Job drawing, mm, ordinate dimensions from the low corner. One solid piece. Round coordinates to 2 decimals unless told otherwise and drop trailing zeros. Order: outer loops, then holes, each group sorted by start corner. A loop starts at its lowest first (then second) coordinate and runs counter-clockwise, first axis right, second up. Notation, with made-up numbers: M 41,70.5 L 86,70.5 A13 ccw 86,84.5 Z; hole C 39.5,59 d1. An arc over 180 degrees is marked long. Answer as a JSON object with one key per item and string values. Group by question number.
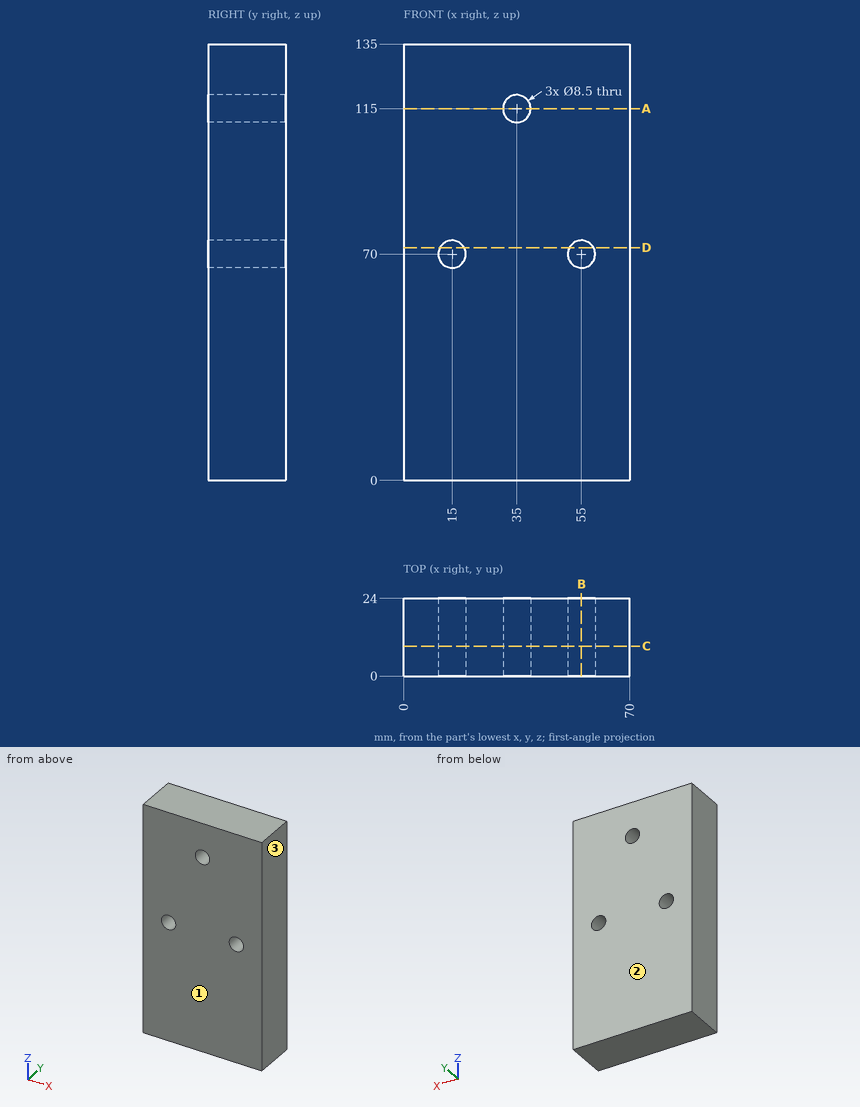
Item 1: Flat gauge pin, fed straight in: pin 1 Ø10 at (x, z) = (55, 70) entering from +Y. Where does the tip first touch, or does it go through?
Item 2: Two-plate mould, pull along Y, no slides. Class the marked faces 1, 2 and 3: +Y half, -Y half, draft (parallel to the pull), parting line (faces both ways), or undercut.
Item 3: Cut at D-D, the plane z = 72. Give the cut face in (x, y), and give its area (3 significant figures).
Item 4: Drill centre lines: line 1 (X direction, y = 11.5, z = 70); line 2 (Z direction, x = 55, y = 16); line 3 (Z direction, x = 34.5, y = 20.25). Where is each one in solid material? Low to high. Write a range as [from, to].
Item 5: Cut at A-A, the plane z = 115. Give the cut face in (x, y).
Item 6: Cut at C-C, the plane y = 9.25. Give the cut face in (x, z).
Item 7: Cut at B-B, the plane x = 55. Give the cut face in (y, z), and give its area (3 significant figures).
Response values:
{
 "1": {"pin 1": "y = 24"},
 "2": {"face 1": "-Y half", "face 2": "+Y half", "face 3": "draft"},
 "3": {"outline": "M 0,0 L 11.25,0 L 11.25,24 L 0,24 Z; M 18.75,0 L 51.25,0 L 51.25,24 L 18.75,24 Z; M 58.75,0 L 70,0 L 70,24 L 58.75,24 Z", "area": "1,320 mm^2"},
 "4": {"line 1": "[0, 10.75], [19.25, 50.75], [59.25, 70]", "line 2": "[0, 65.75], [74.25, 135]", "line 3": "[0, 110.78], [119.22, 135]"},
 "5": {"outline": "M 0,0 L 30.75,0 L 30.75,24 L 0,24 Z; M 39.25,0 L 70,0 L 70,24 L 39.25,24 Z"},
 "6": {"outline": "M 0,0 L 70,0 L 70,135 L 0,135 Z; hole C 15,70 d8.5; hole C 35,115 d8.5; hole C 55,70 d8.5"},
 "7": {"outline": "M 0,0 L 24,0 L 24,65.75 L 0,65.75 Z; M 0,74.25 L 24,74.25 L 24,135 L 0,135 Z", "area": "3,040 mm^2"}
}
